Source: CAD feature listing. Evaluate the final solid. Frame: model axes, mm. Face numbers are marked on the shaded views. A direction names the side the tool comes from. Give positions to 0.01 mm unless a question says otherwise; leave off trailing zeros. Write each loop counter-clockwise with the first axis right and the second up, starting at its lowest first coordinate (ties: lowest second). Pieces come first, ordered by that corner, then holes. Notation, with made-up numbers: (-19, -35) -> (35, -35) arc R24 cw to (35, 4) -> close; hole circle Ø11 at (67.25, 47.5). An arc over 180 degrees is marked (long way). Use one line per item in the form item = value. Start each with the question number.
(1) Cut plane B-B, the plane y = 72.5. Output: boundary loops of the cut face in (x, z), and give its area (3 significant figures).
(2) Cut plane C-C, the plane y = 0. Output: boundary loops of the cut face in (x, z).
(3) Draft query along Y for the marked faces 3, 4 and 5. Return one class per face: pulls with the +Y half, pulls with the -Y half, needs draft (parallel to the pull), parting line crosses it, or undercut.
(4) Material intervals for line 1 along Y through (x, z) = (-70, 29); line 2 along Z through (x, y) = (43, -57); line 3 along Y through (x, z) = (-67, 40), sorted ascending. Write a range as from..to.
(5) Cut plane A-A, the plane z = 7. Output: boundary loops of the cut face in (x, y).
(6) First-contact query: P1, Ø8, axis at x = -42, z = 46, coming from the +Y side; P2, Ø19.5, axis at x = -70, y = 70, coming from the +Z side. Flat tips, straight axial feed; report the tip coordinate or a pass-through.
(7) Cut plane D-D, the plane x = -16. Output: boundary loops of the cut face in (y, z).
(8) Set-up query: the marked faces 1 and 2. Return all of +Z, -Z, +X, -X, +Y, -Y with unobstructed straight access to the full face (end or side cutting, diameter ignored); none if empty.
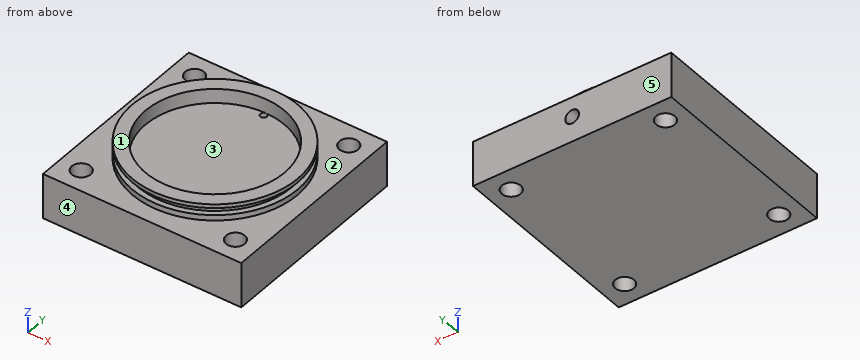
from build123d import *

# Parameters (mm, degrees)
SKETCH_1_W               = 180
SKETCH_1_H               = 180
EXTRUDE_1_DEPTH          = 41
SKETCH_2_R               = 75
EXTRUDE_2_DEPTH          = 15
SKETCH_3_R               = 63
CUT_EXTRUDE_1_DEPTH      = 13
SKETCH_4_W               = 6.5
SKETCH_4_H               = 5
CUT_EXTRUDE_2_REACH      = 136.347
CUT_EXTRUDE_2_END_RADIUS = 5.5626
SKETCH_9_R               = 3
CUT_EXTRUDE_4_REACH      = 141.054
SKETCH_11_R              = 8.5


with BuildPart() as part:
    # 草图1 → 凸台-拉伸1 (new body)
    with BuildSketch(Plane.XY):
        Rectangle(SKETCH_1_W, SKETCH_1_H)
    extrude(amount=EXTRUDE_1_DEPTH)

    # 草图2 → 凸台-拉伸2 (add)
    with BuildSketch(Plane.XY.offset(41)):
        Circle(SKETCH_2_R)
    extrude(amount=EXTRUDE_2_DEPTH)

    # 草图3 → 切除-拉伸1 (cut)
    with BuildSketch(Plane.XY.offset(56)):
        Circle(SKETCH_3_R)
    extrude(amount=-CUT_EXTRUDE_1_DEPTH, mode=Mode.SUBTRACT)

    # 草图4 → 切除-旋转1 (revolve, cut)
    with BuildSketch(Plane(origin=(0, 0, 0), x_dir=(0, 0, -1), z_dir=(1, 0, 0)), mode=Mode.PRIVATE) as cut_revolve_1_sk:
        with Locations((-49.25, 72.5)):
            Rectangle(SKETCH_4_W, SKETCH_4_H)
    revolve(cut_revolve_1_sk.sketch.rotate(Axis((0, 0, 56), (0, 0, -1)), 90), axis=Axis((0, 0, 56), (0, 0, -1)), mode=Mode.SUBTRACT)

    # 草图6 → 1/4 NPT 螺纹孔1 (revolve, cut)
    with BuildSketch(Plane(origin=(0, 90, 23), x_dir=(0, 0, 1), z_dir=(1, 0, 0))):
        Polygon((0, 0), (0, 36.342347279), (5.5626, 33), (5.5626, 10.02), (5.943676082, 10.02), (6.2436883, 0), align=None)
    revolve(axis=Axis((0, 96.35, 23), (0, -1, 0)), mode=Mode.SUBTRACT)

    # 切除-拉伸2: up to this cylinder (the profile starts outside it)
    cut_extrude_2_end = Plane(origin=(0, 60, 23), z_dir=(0, 1, 0)) * Cylinder(CUT_EXTRUDE_2_END_RADIUS, 284.8192, mode=Mode.PRIVATE)
    # 草图9 → 切除-拉伸2 (cut, up to the surface)
    with BuildSketch(Plane.XY.offset(43), mode=Mode.PRIVATE) as cut_extrude_2_sk1:
        with Locations(Location((0, 60, 0), (0, 0, 270))):
            Circle(SKETCH_9_R)
    cut_extrude_2_tool1 = extrude(cut_extrude_2_sk1.sketch, amount=-CUT_EXTRUDE_2_REACH, mode=Mode.PRIVATE) - cut_extrude_2_end
    add(cut_extrude_2_tool1.solids().sort_by_distance((0, 60, 43))[0], mode=Mode.SUBTRACT)

    # 草图11 → 切除-拉伸4 (cut, up to next)
    with BuildSketch(Plane(origin=(0, 0, 0), x_dir=(-1, 0, 0), z_dir=(0, 0, -1)), mode=Mode.PRIVATE) as cut_extrude_4_sk1:
        with Locations((-70, 70)):
            Circle(SKETCH_11_R)
    cut_extrude_4_tool1 = extrude(cut_extrude_4_sk1.sketch, amount=-CUT_EXTRUDE_4_REACH, mode=Mode.PRIVATE) & part.part
    # 草图11 → 切除-拉伸4 (cut, up to next)
    with BuildSketch(Plane(origin=(0, 0, 0), x_dir=(-1, 0, 0), z_dir=(0, 0, -1)), mode=Mode.PRIVATE) as cut_extrude_4_sk2:
        with Locations((70, 70)):
            Circle(SKETCH_11_R)
    cut_extrude_4_tool2 = extrude(cut_extrude_4_sk2.sketch, amount=-CUT_EXTRUDE_4_REACH, mode=Mode.PRIVATE) & part.part
    # 草图11 → 切除-拉伸4 (cut, up to next)
    with BuildSketch(Plane(origin=(0, 0, 0), x_dir=(-1, 0, 0), z_dir=(0, 0, -1)), mode=Mode.PRIVATE) as cut_extrude_4_sk3:
        with Locations((70, -70)):
            Circle(SKETCH_11_R)
    cut_extrude_4_tool3 = extrude(cut_extrude_4_sk3.sketch, amount=-CUT_EXTRUDE_4_REACH, mode=Mode.PRIVATE) & part.part
    # 草图11 → 切除-拉伸4 (cut, up to next)
    with BuildSketch(Plane(origin=(0, 0, 0), x_dir=(-1, 0, 0), z_dir=(0, 0, -1)), mode=Mode.PRIVATE) as cut_extrude_4_sk4:
        with Locations((-70, -70)):
            Circle(SKETCH_11_R)
    cut_extrude_4_tool4 = extrude(cut_extrude_4_sk4.sketch, amount=-CUT_EXTRUDE_4_REACH, mode=Mode.PRIVATE) & part.part
    add(cut_extrude_4_tool1.solids().sort_by_distance((70, 70, 0))[0], mode=Mode.SUBTRACT)
    add(cut_extrude_4_tool2.solids().sort_by_distance((-70, 70, 0))[0], mode=Mode.SUBTRACT)
    add(cut_extrude_4_tool3.solids().sort_by_distance((-70, -70, 0))[0], mode=Mode.SUBTRACT)
    add(cut_extrude_4_tool4.solids().sort_by_distance((70, -70, 0))[0], mode=Mode.SUBTRACT)


solid = part.part
Geometry says:
q1.outline = (-90, 0) -> (-78.12, 0) -> (-78.12, 41) -> (-90, 41) -> close; (-61.88, 0) -> (61.88, 0) -> (61.88, 41) -> (19.2, 41) -> (19.2, 46) -> (-19.2, 46) -> (-19.2, 41) -> (-61.88, 41) -> close; (-19.2, 52.5) -> (19.2, 52.5) -> (19.2, 56) -> (-19.2, 56) -> close; (78.12, 0) -> (90, 0) -> (90, 41) -> (78.12, 41) -> close; hole circle Ø11.13 at (0, 23)
q1.area = 6,280 mm^2
q2.outline = (-90, 0) -> (90, 0) -> (90, 41) -> (75, 41) -> (75, 46) -> (70, 46) -> (70, 52.5) -> (75, 52.5) -> (75, 56) -> (63, 56) -> (63, 43) -> (-63, 43) -> (-63, 56) -> (-75, 56) -> (-75, 52.5) -> (-70, 52.5) -> (-70, 46) -> (-75, 46) -> (-75, 41) -> (-90, 41) -> close
q3.face_3 = undercut
q3.face_4 = pulls with the -Y half
q3.face_5 = pulls with the +Y half
q4.line_1 = -90..-78.5, -61.5..61.5, 78.5..90
q4.line_2 = 0..46, 52.5..56
q4.line_3 = -90..-77.95, -62.05..62.05, 77.95..90
q5.outline = (-90, -90) -> (90, -90) -> (90, 90) -> (-90, 90) -> close; hole circle Ø17 at (-70, -70); hole circle Ø17 at (-70, 70); hole circle Ø17 at (70, -70); hole circle Ø17 at (70, 70)
q6.P1 = 64.66
q6.P2 = 41
q7.outline = (-90, 0) -> (90, 0) -> (90, 41) -> (73.27, 41) -> (73.27, 46) -> (68.15, 46) -> (68.15, 52.5) -> (73.27, 52.5) -> (73.27, 56) -> (60.93, 56) -> (60.93, 43) -> (-60.93, 43) -> (-60.93, 56) -> (-73.27, 56) -> (-73.27, 52.5) -> (-68.15, 52.5) -> (-68.15, 46) -> (-73.27, 46) -> (-73.27, 41) -> (-90, 41) -> close
q8.face_1 = +Z, +X, -X, +Y, -Y
q8.face_2 = +Z
